The listing builds one solid part. Answer for the finished solid, in the listing's coordinates (mm). A direction names the side the tool comes from. Give positions to 0.01 mm unless a question says otherwise; leave off trailing zeros. Loops run counter-clockwise (first coordinate to the right, second up) from the corner with the lowest first, then second, coordinate; pieces in that order, holes last. Notation, with made-up numbers: M -9,16 L 12,16 A28 ccw 12,54 Z; hole C -28,20.25 d7. An arc over 180 degrees is marked long. One line per item, written item: value. Start each with the question number.
Q1. For faces 4 (the cylindrical face through (43.748, 10.099, 1.775)), 5 (the cylindrical face through (11.27, 8.5, 2.66)), 6 (the flat face through (43, 8, 3.6)), determine the directions among +Z, -Z, +X, -X, +Y, -Y from which every point of the face is accessible in a straight line to the end or side of a thin tool.
Q2. Consider L1, parallel to X at y = 13, z = 6; L2, parallel to Y at x = 18.5, z = 2.4; L3, parallel to X at y = 8, z = 2.25. Determine where each line is inside the solid, lowest interval first.
Q3. A cutting plane is placed at B-B, the plane z = 7.25. Determine the outline of the cut face in (x, y).
Q4. A cutting plane is placed at D-D, the plane x = 18.5. Determine the outline of the cut face in (y, z), and give its area (3 significant figures).
Q5. A cutting plane is placed at A-A, the plane x = 53.5. Determine the outline of the cut face in (y, z).
Q6. The mould has two halves that part along Y. Classify faces 1 (the flat face through (30, 10, 0)), 2 (the cylindrical face through (37.504, 10.176, 5.831)), 3 (the flat face through (30, 0, 4)): +Y half, -Y half, draft (parallel to the pull), parting line (faces both ways), or undercut.
Q7. Flat-ended cylindrical pins translate along their axes: pin 1 (5 mm diameter, centred on x = 6.5, y = 10, fed in from -Z); pin 2 (3 mm diameter, centred on x = 6, y = 11.5, fed in from -Z); pin 3 (6.5 mm diameter, centred on x = 41.5, y = 10, fed in from +Z). Find the tip coordinate at first contact, or state that the pin passes through.
Q8. A cutting plane is placed at C-C, the plane y = 10. State how many separate pieces and enclosed holes the cut face has, and give its area (3 significant figures).
from build123d import *

# Parameters (mm, degrees)
SKETCH1_W                                           = 60
SKETCH1_H                                           = 20
BOSS_EXTRUDE1_DEPTH                                 = 8
CBORE_FOR_M4_HEX_SOCKET_HEAD_CAP_SCREW2_D           = 4.5
CBORE_FOR_M4_HEX_SOCKET_HEAD_CAP_SCREW2_CBORE_D     = 8
CBORE_FOR_M4_HEX_SOCKET_HEAD_CAP_SCREW2_CBORE_DEPTH = 4.4
CBORE_FOR_M5_HEX_SOCKET_HEAD_CAP_SCREW1_D           = 5.5
CBORE_FOR_M5_HEX_SOCKET_HEAD_CAP_SCREW1_CBORE_D     = 10
CBORE_FOR_M5_HEX_SOCKET_HEAD_CAP_SCREW1_CBORE_DEPTH = 5.4
CHAMFER1_SIZE                                       = 2


with BuildPart() as part:
    # Sketch1 → Boss-Extrude1 (new body)
    with BuildSketch(Plane.XY):
        with Locations((30, 10)):
            Rectangle(SKETCH1_W, SKETCH1_H)
    extrude(amount=BOSS_EXTRUDE1_DEPTH)

    # CBORE for M4 Hex Socket Head Cap Screw2 (through all)
    with Locations(Plane.XY.offset(8)):
        with Locations((41.5, 10), (18.5, 10)):
            CounterBoreHole(CBORE_FOR_M4_HEX_SOCKET_HEAD_CAP_SCREW2_D / 2, CBORE_FOR_M4_HEX_SOCKET_HEAD_CAP_SCREW2_CBORE_D / 2, CBORE_FOR_M4_HEX_SOCKET_HEAD_CAP_SCREW2_CBORE_DEPTH)

    # CBORE for M5 Hex Socket Head Cap Screw1 (through all)
    with Locations(Plane(origin=(0, 0, 0), x_dir=(1, 0, 0), z_dir=(0, 0, -1))):
        with Locations((53.5, -10), (6.5, -10)):
            CounterBoreHole(CBORE_FOR_M5_HEX_SOCKET_HEAD_CAP_SCREW1_D / 2, CBORE_FOR_M5_HEX_SOCKET_HEAD_CAP_SCREW1_CBORE_D / 2, CBORE_FOR_M5_HEX_SOCKET_HEAD_CAP_SCREW1_CBORE_DEPTH)

    # Chamfer1
    chamfer1_edges = [part.edges().sort_by_distance(p)[0] for p in [
        (0, 20, 4),
        (60, 20, 4),
        (60, 0, 4),
        (0, 0, 4),
    ]]
    chamfer(chamfer1_edges, length=CHAMFER1_SIZE)


solid = part.part
Answer block:
1. face 4: +Z, -Z
1. face 5: -Z
1. face 6: +Z
2. L1: 0 to 15.85, 21.15 to 38.85, 44.15 to 60
2. L2: 0 to 7.75, 12.25 to 20
2. L3: 0 to 1.92, 11.08 to 17.47, 19.53 to 40.47, 42.53 to 48.92, 58.08 to 60
3. outline: M 0,2 L 2,0 L 58,0 L 60,2 L 60,18 L 58,20 L 2,20 L 0,18 Z; hole C 6.5,10 d5.5; hole C 18.5,10 d8; hole C 41.5,10 d8; hole C 53.5,10 d5.5
4. outline: M 0,0 L 7.75,0 L 7.75,3.6 L 6,3.6 L 6,8 L 0,8 Z; M 12.25,0 L 20,0 L 20,8 L 14,8 L 14,3.6 L 12.25,3.6 Z
4. area: 109 mm^2
5. outline: M 0,0 L 5,0 L 5,5.4 L 7.25,5.4 L 7.25,8 L 0,8 Z; M 12.75,5.4 L 15,5.4 L 15,0 L 20,0 L 20,8 L 12.75,8 Z
6. face 1: draft
6. face 2: undercut
6. face 3: -Y half
7. pin 1: through
7. pin 2: z = 5.4
7. pin 3: z = 3.6
8. separate pieces: 5
8. enclosed holes: 0
8. area: 241 mm^2
